```python
from build123d import *

# Parameters (mm, degrees)
MOUNTING_START               = -7.5
MOUNTING_FLANGE_SKETCH_R     = 37.5
MOUNTING_FLANGE_SKETCH_R_2   = 7.5
MOUNTING_FLANGE_3_LUGS_DEPTH = 7.5


with BuildPart() as part:
    # Housing Profile Sketch → Housing Sleeve Revolve (revolve)
    with BuildSketch(Plane.XY):
        Polygon((45, 0), (37.5, 0), (37.5, 70), (45, 70), (45, 55), (42, 55), (42, 45), (45, 45), (45, 25), (42, 25), (42, 15), (45, 15), align=None)
    revolve(axis=Axis((0, -100.894385012, 0), (0, 1, 0)))

    # Mounting Flange Sketch → Mounting Flange 3 Lugs (add)
    with BuildSketch(Plane.XZ.offset(MOUNTING_START)):
        with BuildLine():
            ThreePointArc((-26.98330478, 53.646097371), (-52.004825497, 30.025), (-59.950535527, -3.454821269))
            ThreePointArc((-59.950535527, -3.454821269), (-62.126875731, -13.743136068), (-69.221670101, -21.50520866))
            ThreePointArc((-69.221670101, -21.50520866), (-74.521485996, -43.025), (-53.234892064, -49.19512047))
            ThreePointArc((-53.234892064, -49.19512047), (-42.965342828, -46.931884607), (-32.967230748, -50.191276103))
            ThreePointArc((-32.967230748, -50.191276103), (0, -60.05), (32.967230748, -50.191276103))
            ThreePointArc((32.967230748, -50.191276103), (42.965342828, -46.931884607), (53.234892064, -49.19512047))
            ThreePointArc((53.234892064, -49.19512047), (74.521485996, -43.025), (69.221670101, -21.50520866))
            ThreePointArc((69.221670101, -21.50520866), (62.126875731, -13.743136068), (59.950535527, -3.454821269))
            ThreePointArc((59.950535527, -3.454821269), (52.004825497, 30.025), (26.98330478, 53.646097371))
            ThreePointArc((26.98330478, 53.646097371), (19.161532903, 60.675020674), (15.986778038, 70.70032913))
            ThreePointArc((15.986778038, 70.70032913), (0, 86.05), (-15.986778038, 70.70032913))
            ThreePointArc((-15.986778038, 70.70032913), (-19.161532903, 60.675020674), (-26.98330478, 53.646097371))
        make_face()
        Circle(MOUNTING_FLANGE_SKETCH_R, mode=Mode.SUBTRACT)
        with Locations((0, 70.05)):
            Circle(MOUNTING_FLANGE_SKETCH_R_2, mode=Mode.SUBTRACT)
        with Locations((60.665079535, -35.025)):
            Circle(MOUNTING_FLANGE_SKETCH_R_2, mode=Mode.SUBTRACT)
        with Locations((-60.665079535, -35.025)):
            Circle(MOUNTING_FLANGE_SKETCH_R_2, mode=Mode.SUBTRACT)
    extrude(amount=MOUNTING_FLANGE_3_LUGS_DEPTH)


solid = part.part
```
Read the model definition and answer for the solid it produces. Units are mm, in the model's axes. A direction names the side the tool comes from. Give positions to 0.01 mm unless a question says otherwise; leave off trailing zeros. Write each loop counter-clockwise with the first axis right and the second up, starting at its lowest first coordinate (ties: lowest second). Pieces come first, ordered by that corner, then holes. Notation, with made-up numbers: M -20,-32.75 L 11,-32.75 A21 ccw 11,-20.75 Z; hole C 77,-35.75 d5. An arc over 180 degrees is marked long. Put each result on its own line as item: value. Start each with the question number.
1. The part is cut by section C-C, the plane y = 5.5. Give the vertices of the cut face in (x, z) (3 decimals).
2. The part is cut by section A-A, the plane x = 0. Give the number of separate pieces and of enclosed holes in the cut face, and give its area (3 significant figures).
3. For a pull along Z with two mould halves and no side action, classify faces 4 (the cylindrical face through (53.172, 3.802, -34.695)), 5 (the cylindrical face through (40.06, 49.93, -12.62)), 6 (the flat face through (-23, 0, 30)) as released by +Z, released by -Z, zero draft, split by the parting line, or undercut.
4. Each of these flat-tipped pins is pushed along its axis until it touches: pin 1 Ø3 at (x, z) = (55.5, -26.5) entering from +Y; pin 2 Ø1 at (x, z) = (30, -18.5) entering from -Y; pin 3 Ø19.5 at (x, z) = (-60.67, -35.02) entering from -Y; pin 4 Ø4 at (x, y) = (-41, 39.5) entering from +Z. Where does it stop, or does it pass through?
5. Which of the six approach directions +Z, -Z, +X, -X, +Y, -Y give full straight-line access (tool end or side, diameter ignored) to faces 1 (the flat face through (-40, 45, -14)), 2 (the flat face through (-29, 7.5, 35)), 3 (the cylindrical face through (-19.08, 3.8, 60.8))?
6. Consider line 1 along Z through (x, y) = (0, 3.5); line 2 along X through (y, z) = (43, 0); line 3 along X through (y, z) = (47.5, 0). Determine where each line is inside the solid, lowest interval first.
7. The part is cut by section B-B, the plane z = 0. Give the vertices of the cut face in (x, y), and give its area (3 significant figures).
8. The part is cut by section D-D, the plane y = 17. Give the vertices of the cut face in (x, z), and give its area (3 significant figures).
Final values:
1. outline: M -69.222,-21.505 A16 ccw -53.235,-49.195 A20 cw -32.967,-50.191 A60.05 ccw 32.967,-50.191 A20 cw 53.235,-49.195 A16 ccw 69.222,-21.505 A20 cw 59.951,-3.455 A60.05 ccw 26.983,53.646 A20 cw 15.987,70.7 A16 ccw -15.987,70.7 A20 cw -26.983,53.646 A60.05 ccw -59.951,-3.455 A20 cw Z; hole C -60.665,-35.025 d15; hole C 0,0 d75; hole C 0,70.05 d15; hole C 60.665,-35.025 d15
2. separate pieces: 3
2. enclosed holes: 0
2. area: 1,240 mm²
3. face 4: undercut
3. face 5: split by the parting line
3. face 6: zero draft
4. pin 1: stops at y = 7.5
4. pin 2: passes through
4. pin 3: stops at y = 0
4. pin 4: stops at z = 22.45
5. face 1: none
5. face 2: +Y
5. face 3: +Z, -X, +Y, -Y
6. line 1: z = -60.05 to -37.5, 37.5 to 62.55, 77.55 to 86.05
6. line 2: x = -45 to -37.5, 37.5 to 45
6. line 3: x = -42 to -37.5, 37.5 to 42
7. outline: M -60.05,0 L -37.5,0 L -37.5,70 L -45,70 L -45,55 L -42,55 L -42,45 L -45,45 L -45,25 L -42,25 L -42,15 L -45,15 L -45,7.5 L -60.05,7.5 Z; M 37.5,0 L 60.05,0 L 60.05,7.5 L 45,7.5 L 45,15 L 42,15 L 42,25 L 45,25 L 45,45 L 42,45 L 42,55 L 45,55 L 45,70 L 37.5,70 Z
7. area: 1,160 mm²
8. outline: C 0,0 d84; hole C 0,0 d75
8. area: 1,120 mm²
